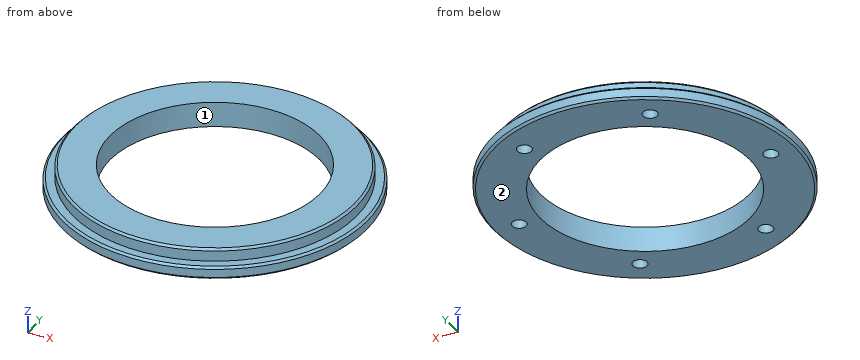
from build123d import *

# Parameters (mm, degrees)
SKETCH1_R             = 72.5
SKETCH1_R_2           = 50
BOSS_EXTRUDE1_DEPTH   = 6
SKETCH2_R             = 67.5
SKETCH2_R_2           = 50
BOSS_EXTRUDE2_DEPTH   = 6
CHAMFER1_SIZE         = 1
SKETCH3_R             = 3
CUT_EXTRUDE1_DEPTH    = 8
M8_TAPPED_HOLE1_D     = 6.8
M8_TAPPED_HOLE1_DEPTH = 8
M8_TAPPED_HOLE1_TIP   = 2.042926105


with BuildPart() as part:
    # Sketch1 → Boss-Extrude1 (new body)
    with BuildSketch(Plane.XY):
        Circle(SKETCH1_R)
        Circle(SKETCH1_R_2, mode=Mode.SUBTRACT)
    extrude(amount=BOSS_EXTRUDE1_DEPTH)

    # Sketch2 → Boss-Extrude2 (add)
    with BuildSketch(Plane.XY.offset(6)):
        Circle(SKETCH2_R)
        Circle(SKETCH2_R_2, mode=Mode.SUBTRACT)
    extrude(amount=BOSS_EXTRUDE2_DEPTH)

    # Chamfer1
    chamfer1_edges = [part.edges().sort_by_distance(p)[0] for p in [
        (-67.5, 0, 12),
        (-72.5, 0, 0),
        (-72.5, 0, 6),
    ]]
    chamfer(chamfer1_edges, length=CHAMFER1_SIZE)

    # Sketch3 → Cut-Extrude1 (cut)
    with BuildSketch(Plane(origin=(0, 0, 0), x_dir=(-1, 0, 0), z_dir=(0, 0, -1))):
        with Locations((-30, 51.961524227)):
            Circle(SKETCH3_R)
        with Locations((-60, 0)):
            Circle(SKETCH3_R)
        with Locations((30, 51.961524227)):
            Circle(SKETCH3_R)
        with Locations((60, 0)):
            Circle(SKETCH3_R)
        with Locations((30, -51.961524227)):
            Circle(SKETCH3_R)
        with Locations((-30, -51.961524227)):
            Circle(SKETCH3_R)
    extrude(amount=-CUT_EXTRUDE1_DEPTH, mode=Mode.SUBTRACT)

    # M8 Tapped Hole1
    with Locations(Plane(origin=(0, 0, 0), x_dir=(-1, 0, 0), z_dir=(0, 0, -1))):
        with Locations((-30, 51.961524227), (30, 51.961524227), (60, 0), (30, -51.961524227), (-30, -51.961524227), (-60, 0)):
            Hole(M8_TAPPED_HOLE1_D / 2, depth=M8_TAPPED_HOLE1_DEPTH)
            with Locations((0, 0, -(M8_TAPPED_HOLE1_DEPTH + M8_TAPPED_HOLE1_TIP / 2))):  # 118° drill point
                Cone(0, M8_TAPPED_HOLE1_D / 2, M8_TAPPED_HOLE1_TIP, mode=Mode.SUBTRACT)


solid = part.part
Check sheet for the modelled part. Datum: model origin and axes. Units: mm. Face numbers are marked on the shaded views. Give positions to 0.01 mm unless a question says otherwise; leave off trailing zeros. Write each loop counter-clockwise with the first axis right and the second up, starting at its lowest first coordinate (ties: lowest second). Pieces come first, ordered by that corner, then holes. Notation, with made-up numbers: M 64,-24.75 L 98,-24.75 A28 ccw 98,-4.75 Z; hole C -10.5,63 d6. An arc over 180 degrees is marked long. Use one line per item in the form item = value.
(1) Draft check along Y on the marked faces 1 and 2. Enter one of: pulls with the +Y half, pulls with the -Y half, needs draft (parallel to the pull), parting line crosses it, or undercut.
Answer block:
face_1 = undercut
face_2 = needs draft
(2) Section check A-A on x = 0. Record the boundary of the cut face in (y, z), plus the area to 3 significant figures.
Answer block:
outline = M -72.5,1 L -71.5,0 L -50,0 L -50,12 L -66.5,12 L -67.5,11 L -67.5,6 L -71.5,6 L -72.5,5 Z; M 50,0 L 71.5,0 L 72.5,1 L 72.5,5 L 71.5,6 L 67.5,6 L 67.5,11 L 66.5,12 L 50,12 Z
area = 477 mm2
(3) Depth check by flat-ended pin: P1, Ø1, axis at x = -48, z = 2, coming from the +Y side; P2, Ø4, axis at y = 46.5, z = 1.5, coming from the +X side; P3, Ø6, axis at x = -39.5, z = 10, coming from the -Y side. Enter the tip coordinate at first touch or a pass-through.
Answer block:
P1 = 54.77
P2 = 57.24
P3 = -56.78
(4) Material ranges on line 1 along Y through (x, z) = (-30, 3); line 2 along Y through (x, z) = (-28.5, 8.5); line 3 along Y through (x, z) = (36, 5.25), recorded low to high.
Answer block:
line_1 = -66 to -55.36, -48.56 to -40, 40 to 48.56, 55.36 to 66
line_2 = -61.19 to -54.05, -49.88 to -41.08, 41.08 to 49.88, 54.05 to 61.19
line_3 = -62.64 to -34.7, 34.7 to 62.64
